Source: three-view drawing plus pictorial views. Frame: mm from the lowest corner of the part. Give positions to 0.01 mm unless a question says otherwise; leave off trailing zeros. Loops run counter-clockwise (first coordinate to the right, second up) from the corner with the lowest first, then second, coordinate; pieces in that order, holes last. Notation, with made-up numbers: (29, 76.5) -> (50, 76.5) arc R18 cw to (50, 107.5) -> close; hole circle Ø8 at (9.25, 27). An arc over 180 degrees is marked (long way). Put each result on its own line as item: value.
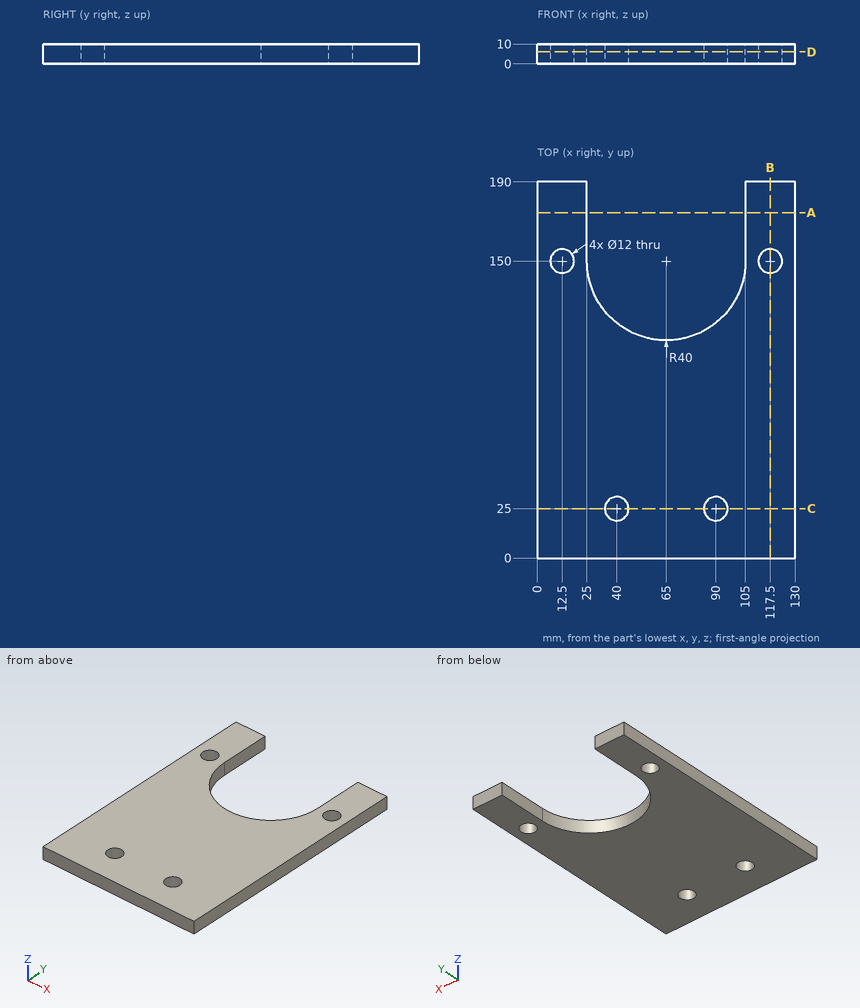
(1) Section A-A on y = 174.5. Return loops of the section in (x, z).
Calculated:
outline: (0, 0) -> (25, 0) -> (25, 10) -> (0, 10) -> close; (105, 0) -> (130, 0) -> (130, 10) -> (105, 10) -> close
(2) Section B-B on x = 117.5. Return loops of the section in (y, z), then the cut area to 3 significant figures.
Calculated:
outline: (0, 0) -> (144, 0) -> (144, 10) -> (0, 10) -> close; (156, 0) -> (190, 0) -> (190, 10) -> (156, 10) -> close
area: 1,780 mm²
(3) Line query: probe 1 along X at (y, z) = (150.5, 8.5); probe 2 along Y at (x, z) = (12.5, 8.25); probe 3 along X at (y, z) = (26, 5.75). Output: solid intervals per line, ascending. Write a range as from..to.
Calculated:
probe 1: x = 0..6.52, 18.48..25, 105..111.52, 123.48..130
probe 2: y = 0..144, 156..190
probe 3: x = 0..34.08, 45.92..84.08, 95.92..130
(4) Section C-C on y = 25. Return loops of the section in (x, z), then the cut area to 3 significant figures.
Calculated:
outline: (0, 0) -> (34, 0) -> (34, 10) -> (0, 10) -> close; (46, 0) -> (84, 0) -> (84, 10) -> (46, 10) -> close; (96, 0) -> (130, 0) -> (130, 10) -> (96, 10) -> close
area: 1,060 mm²
(5) First-contact query: P1, Ø11, axis at x = 117.5, y = 150, coming from the -Z side. Flat tip, straight axial feed; report the tip coordinate or a pass-through.
Calculated:
P1: passes through
(6) Section D-D on z = 6. Return loops of the section in (x, y).
Calculated:
outline: (0, 0) -> (130, 0) -> (130, 190) -> (105, 190) -> (105, 150) arc R40 cw to (25, 150) -> (25, 190) -> (0, 190) -> close; hole circle Ø12 at (12.5, 150); hole circle Ø12 at (40, 25); hole circle Ø12 at (90, 25); hole circle Ø12 at (117.5, 150)
